```python
from build123d import *

# Parameters (mm, degrees)
EXTRUDE_1_DEPTH     = 4
EXTRUDE_1_2_DEPTH   = 4
EXTRUDE_1_3_DEPTH   = 4
SKETCH_2_R          = 90
SKETCH_2_R_2        = 57.5
EXTRUDE_2_DEPTH     = 50
SKETCH_4_R          = 57.5
SKETCH_4_R_2        = 50
EXTRUDE_3_DEPTH     = 100
CUT_EXTRUDE_1_DEPTH = 485.810454508
EXTRUDE_START       = 10
EXTRUDE_4_DEPTH     = 10


with BuildPart() as part:
    # Sketch 1 → Extrude 1 (new, symmetric)
    with BuildSketch(Plane.XY):
        with BuildLine():
            Line((-10.924807901, 55.668937127), (-50.690571005, 338.617043901))
            Line((-50.690571005, 338.617043901), (-206.438031879, 275.690985101))
            Line((-206.438031879, 275.690985101), (-37.918188894, 43.743319974))
            ThreePointArc((-37.918188894, 43.743319974), (-25.199590106, 51.467322598), (-10.924807901, 55.668937127))
        make_face()
    extrude(amount=EXTRUDE_1_DEPTH, both=True)



with BuildPart() as body_2:
    # Sketch 1 → Extrude 1 2 (new, symmetric)
    with BuildSketch(Plane.XY):
        with BuildLine():
            Line((-341.966631122, -58.160848878), (-338.146174396, -79.914727665))
            Line((-338.146174396, -79.914727665), (-308.839134252, -137.932805865))
            Line((-308.839134252, -137.932805865), (-53.490261468, -26.646674297))
            ThreePointArc((-53.490261468, -26.646674297), (-59.462925063, -1.128374922), (-53.490261468, 24.389924453))
            Line((-53.490261468, 24.389924453), (-336.508428621, 6.839151122))
            Line((-336.508428621, 6.839151122), (-341.966631122, -58.160848878))
        make_face()
    extrude(amount=EXTRUDE_1_2_DEPTH, both=True)


with BuildPart() as body_3:
    # Sketch 1 → Extrude 1 3 (new, symmetric)
    with BuildSketch(Plane.XY):
        with BuildLine():
            Line((-14.977351718, -57.136184189), (-46.962925063, -340))
            Line((-46.962925063, -340), (68.037074937, -340))
            Line((68.037074937, -340), (24.752563392, -52.045294277))
            ThreePointArc((24.752563392, -52.045294277), (5.345225431, -58.162057394), (-14.977351718, -57.136184189))
        make_face()
    extrude(amount=EXTRUDE_1_3_DEPTH, both=True)


with BuildPart() as part_1:
    add(part.part)

    add(body_2.part)  # Extrude 2 merges body 2

    add(body_3.part)  # Extrude 2 merges body 3
    # Sketch 2 → Extrude 2 (add, symmetric)
    with BuildSketch(Plane.XY.offset(4)):
        Circle(SKETCH_2_R)
        with Locations((-1.962925063, -1.128374922)):
            Circle(SKETCH_2_R_2, mode=Mode.SUBTRACT)
    extrude(amount=EXTRUDE_2_DEPTH, both=True)

    # Sketch 4 → Extrude 3 (add)
    with BuildSketch(Plane.XY.offset(54)):
        with Locations((-1.962925063, -1.128374922)):
            Circle(SKETCH_4_R)
        with Locations((-1.962925063, -1.128374922)):
            Circle(SKETCH_4_R_2, mode=Mode.SUBTRACT)
    extrude(amount=-EXTRUDE_3_DEPTH)

    # Sketch 7 → Cut-Extrude 1 (cut, through all)
    with BuildSketch(Plane.XY.offset(4)):
        with BuildLine():
            Line((-18.476741558, -88.082972369), (-46.962925063, -340))
            Line((-46.962925063, -340), (68.037074937, -340))
            Line((68.037074937, -340), (29.699950595, -84.958301152))
            ThreePointArc((29.699950595, -84.958301152), (5.825032002, -89.811296629), (-18.476741558, -88.082972369))
        make_face()
    extrude(amount=-CUT_EXTRUDE_1_DEPTH, mode=Mode.SUBTRACT)

    # Sketch 9 → Extrude 4 (add)
    with BuildSketch(Plane.XY.offset(EXTRUDE_START)):
        with BuildLine():
            Line((-206.438031879, -275.690985101), (-56.836712635, -69.782434014))
            ThreePointArc((-56.836712635, -69.782434014), (-37.406446529, -81.858156332), (-15.559269973, -88.644848231))
            Line((-15.559269973, -88.644848231), (-50.690571005, -338.617043901))
            Line((-50.690571005, -338.617043901), (-206.438031879, -275.690985101))
        make_face()
    extrude(amount=-EXTRUDE_4_DEPTH)


solid = part_1.part
```
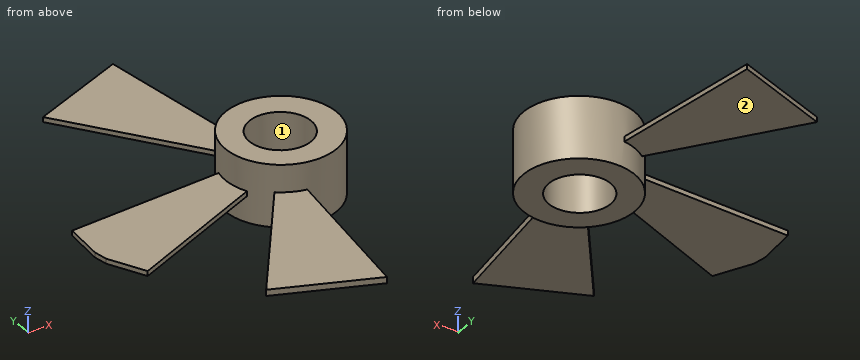
Geometry: final body of the model. Coordinates: model frame, mm. Face numbers are marked on the shaded views. Coordinates: 2 decimals unless noted, no trailing zeros. Order: outer loops, then holes, each group sorted by start corner. A loop starts at its lowest first (then second) coordinate and runs counter-clockwise, first axis right, second up. Notation, with made-up numbers: (-12, -23) -> (2, -23) arc R18 cw to (2, -12) -> close; hole circle Ø5 at (-22.75, 2.5). An arc over 180 degrees is marked (long way). Answer in a Markdown table with one row per item.
Item 1: Section A-A on x = 0. Output: boundary loops of the cut face in (y, z).
Return value:
| item | result |
|---|---|
| outline | (-90, -46) -> (-51.09, -46) -> (-51.09, 54) -> (-90, 54) -> close; (48.83, -46) -> (90, -46) -> (90, 54) -> (48.83, 54) -> close |
Item 2: Section C-C on x = -119. Output: boundary loops of the cut face in (y, z).
Return value:
| item | result |
|---|---|
| outline | (-311.02, 0) -> (-155.34, 0) -> (-155.34, 10) -> (-311.02, 10) -> close; (-55.2, -4) -> (20.33, -4) -> (20.33, 4) -> (-55.2, 4) -> close; (155.34, -4) -> (311.02, -4) -> (311.02, 4) -> (155.34, 4) -> close |
Item 3: Section B-B on y = -105. Output: boundary loops of the cut face in (x, z).
Return value:
| item | result |
|---|---|
| outline | (-325.47, -4) -> (-233.27, -4) -> (-233.27, 4) -> (-325.47, 4) -> close; (-82.42, 0) -> (-17.86, 0) -> (-17.86, 10) -> (-82.42, 10) -> close |
Item 4: Ray query, L1, parallel to Y at x = -41.5, z = 12.5; L2, parallel to X at y = -7, z = -12; L3, parallel to Y at x = -42, z = 32.5. Return the intervals inside material, ascending.
Return value:
| item | result |
|---|---|
| L1 | y = -79.86 to -31.74, 29.48 to 79.86 |
| L2 | x = -89.73 to -51.62, 47.69 to 89.73 |
| L3 | y = -79.6 to -31.08, 28.82 to 79.6 |
Item 5: Contact query for flat-ended pins moving along their axis: P1, Ø3, axis at x = -34.5, z = 40, coming from the -Y side; P2, Ø1.5, axis at x = -35, y = -190, coming from the -Z side; P3, Ø3, axis at x = 20, z = 7.5, coming from the -Y side. Output: stop coordinate, or through.
Return value:
| item | result |
|---|---|
| P1 | stops at y = -83.73 |
| P2 | stops at z = 0 |
| P3 | stops at y = -88.08 |
Item 6: Section D-D on z = -30. Output: boundary loops of the cut face in (x, y), plus the area to 3 significant figures.
Return value:
| item | result |
|---|---|
| outline | circle Ø180 at (0, 0); hole circle Ø100 at (-1.96, -1.13) |
| area | 17,600 mm² |
Item 7: Draft query along X for the marked faces 1 and 2. Return one class per face: released by +X, released by -X, zero draft, split by the parting line, or undercut.
Return value:
| item | result |
|---|---|
| face 1 | undercut |
| face 2 | zero draft |
